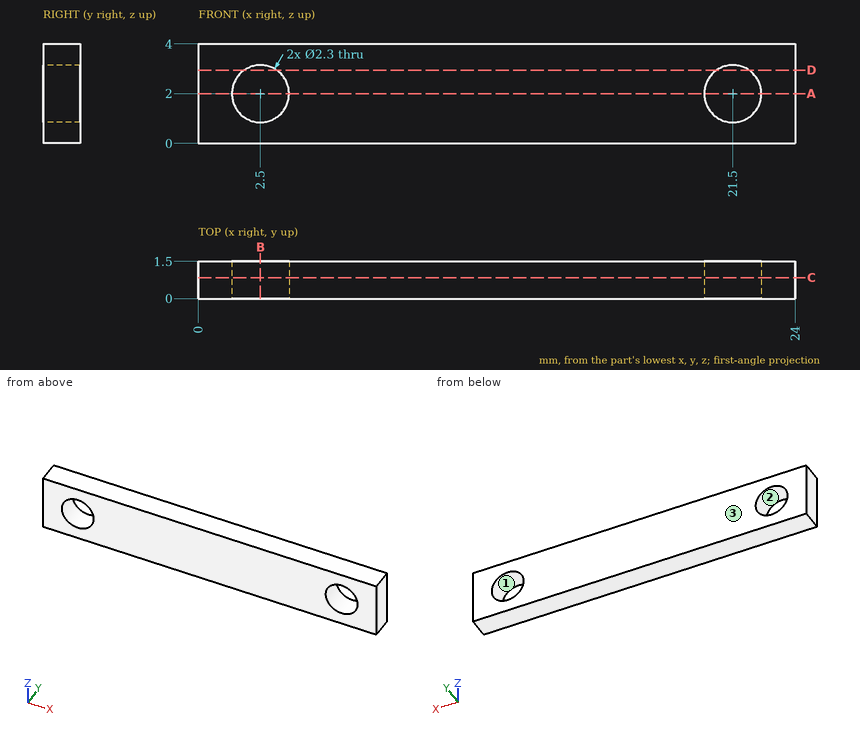
Study the drawing (mm; zero at the part's minimum x, y, z) and answer. Round coordinates to 2 decimals unless told otherwise and drop trailing zeros. Write each loop counter-clockwise with the first axis right and the second up, starting at its lowest first coordinate (ties: lowest second). Pieces come first, ordered by that corner, then holes. Notation, with made-up numbers: (-33, -15) - (-21, -15) arc R23 cw to (-21, 8) - close; hole circle Ø1 at (11, -39.75). An arc over 180 degrees is marked (long way). Use a Markdown table: item, result. Add a question column.
1. The part is cut by section C-C (y = 0.85). Write down the section's boundary in (x, z), and give its area (3 significant figures).
2. For a pull along Z with two mould halves and no side action, classify the marked faces 1, 2 and 3 as +Z half, -Z half, draft (parallel to the pull), parting line (faces both ways), or undercut.
3. The part is cut by section B-B (x = 2.5). Write down the section's boundary in (y, z), and give its area (3 significant figures).
4. Consider line 1 (Z direction, x = 2.5, y = 1); line 2 (X direction, y = 0.4, z = 1.3); line 3 (X direction, y = 1.05, z = 2.9). Determine where each line is inside the solid, lowest interval first.
5. The part is cut by section D-D (z = 2.95). Write down the section's boundary in (x, y).
6. The part is cut by section A-A (z = 2). Write down the section's boundary in (x, y).
Reported:
| question | item | result |
|---|---|---|
| 1 | outline | (0, 0) - (24, 0) - (24, 4) - (0, 4) - close; hole circle Ø2.3 at (2.5, 2); hole circle Ø2.3 at (21.5, 2) |
| 1 | area | 87.7 mm^2 |
| 2 | face 1 | undercut |
| 2 | face 2 | undercut |
| 2 | face 3 | draft |
| 3 | outline | (0, 0) - (1.5, 0) - (1.5, 0.85) - (0, 0.85) - close; (0, 3.15) - (1.5, 3.15) - (1.5, 4) - (0, 4) - close |
| 3 | area | 2.55 mm^2 |
| 4 | line 1 | 0 to 0.85, 3.15 to 4 |
| 4 | line 2 | 0 to 1.59, 3.41 to 20.59, 22.41 to 24 |
| 4 | line 3 | 0 to 1.78, 3.22 to 20.78, 22.22 to 24 |
| 5 | outline | (0, 0) - (1.85, 0) - (1.85, 1.5) - (0, 1.5) - close; (3.15, 0) - (20.85, 0) - (20.85, 1.5) - (3.15, 1.5) - close; (22.15, 0) - (24, 0) - (24, 1.5) - (22.15, 1.5) - close |
| 6 | outline | (0, 0) - (1.35, 0) - (1.35, 1.5) - (0, 1.5) - close; (3.65, 0) - (20.35, 0) - (20.35, 1.5) - (3.65, 1.5) - close; (22.65, 0) - (24, 0) - (24, 1.5) - (22.65, 1.5) - close |
